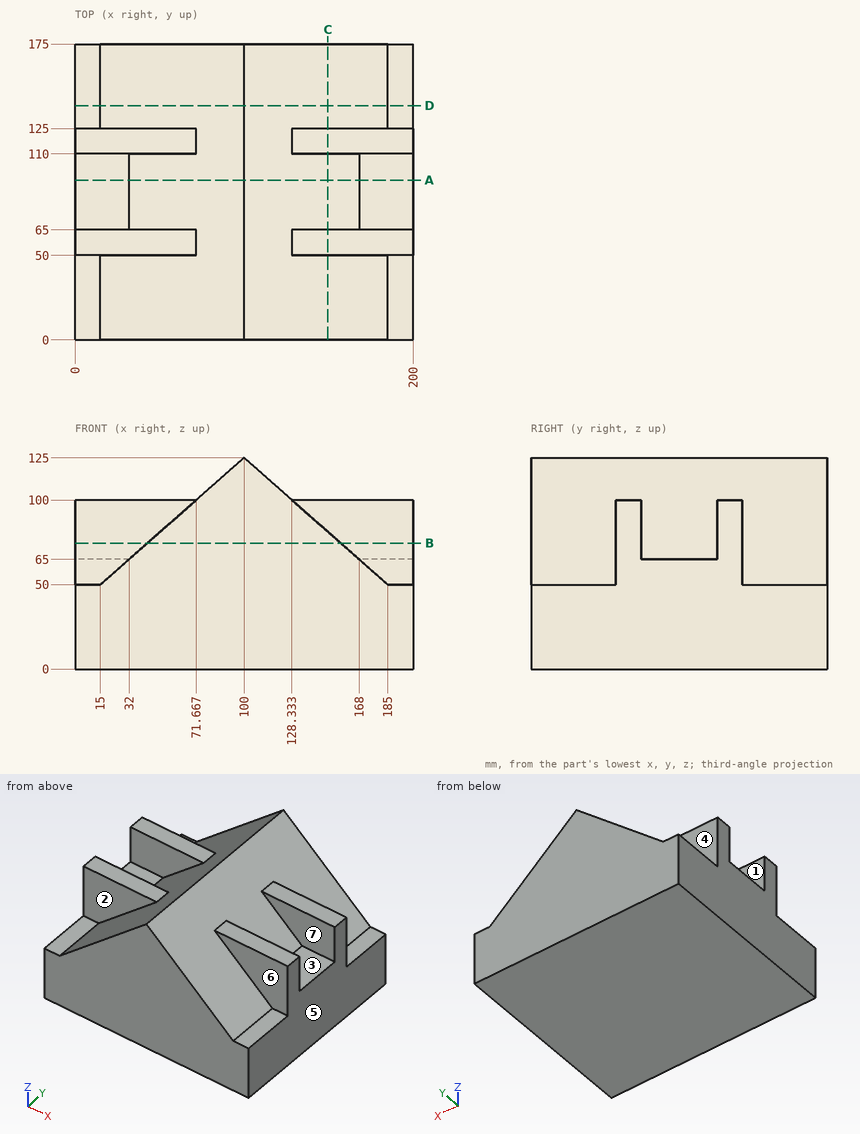
Source: three-view drawing plus pictorial views. Frame: mm from the lowest corner of the part. A direction names the side the tool comes from. Coordinates: 2 decimals unless noted, no trailing zeros. Order: outer loops, then holes, each group sorted by start corner. A loop starts at its lowest first (then second) coordinate and runs counter-clockwise, first axis right, second up. Notation, with made-up numbers: M -4,22 L 4,22 A22 ccw 4,60 Z; hole C 23.25,89.5 d9. An arc over 180 degrees is marked long. One line per question, with ' | ' between items. Start each with the question number.
Item 1: Set-up query: the marked faces 1, 2 and 3. Return all of +Z, -Z, +X, -X, +Y, -Y with unobstructed straight access to the full face (end or side cutting, diameter ignored); none if empty.
Item 2: Ray query, probe 1 along Y at (x, z) = (138.5, 97); probe 2 along Z at (x, y) = (129, 154.5); probe 3 along Z at (x, y) = (26, 68.5). Return the intervals inside material, ascending. Write a range as [from, to].
Item 3: Draft query along Y for the marked faces 4, 5, 6 and 7. Return one class per face: released by +Y, released by -Y, zero draft, split by the parting line, or undercut.
Item 4: Pin query (flat end, axial travel): pin 1 Ø10 at (x, y) = (119.5, 49) entering from +Z (1 decimal); pin 2 Ø10.5 at (x, z) = (172, 83.5) entering from +Y; pin 3 Ø7.5 at (x, y) = (190, 22.5) entering from +Z. Return the tip coordinate at first contact, or that it passes through.
Item 5: Cut plane D-D, the plane y = 138.5. Return the cut outline in (x, z).
Item 6: Cut plane A-A, the plane y = 94.5. Return the cut outline in (x, z), then the cut area to 3 significant figures.
Item 7: Cut plane B-B, the plane z = 74.5. Return the cut outline in (x, y).
Item 8: Cut plane C-C, the plane x = 149.5. Return the cut outline in (y, z), then the cut area to 3 significant figures.
A:
1) face 1: +Z, -X | face 2: +Z, -X, -Y | face 3: +Z, +X
2) probe 1: y = [50, 65], [110, 125] | probe 2: z = [0, 99.41] | probe 3: z = [0, 65]
3) face 4: released by +Y | face 5: zero draft | face 6: released by -Y | face 7: undercut
4) pin 1: stops at z = 112.2 | pin 2: stops at y = 125 | pin 3: stops at z = 50
5) outline: M 0,0 L 200,0 L 200,50 L 185,50 L 100,125 L 15,50 L 0,50 Z
6) outline: M 0,0 L 200,0 L 200,65 L 168,65 L 100,125 L 32,65 L 0,65 Z | area: 17,100 mm2
7) outline: M 0,50 L 42.77,50 L 42.77,0 L 157.23,0 L 157.23,50 L 200,50 L 200,65 L 157.23,65 L 157.23,110 L 200,110 L 200,125 L 157.23,125 L 157.23,175 L 42.77,175 L 42.77,125 L 0,125 L 0,110 L 42.77,110 L 42.77,65 L 0,65 Z
8) outline: M 0,0 L 175,0 L 175,81.32 L 125,81.32 L 125,100 L 110,100 L 110,81.32 L 65,81.32 L 65,100 L 50,100 L 50,81.32 L 0,81.32 Z | area: 14,800 mm2
